Geometry: final body of the model. Coordinates: model frame, mm. A direction names the side the tool comes from. Coordinates: 2 decimals unless noted, no trailing zeros. Order: outer loops, then holes, each group sorted by start corner. A loop starts at its lowest first (then second) coordinate and runs counter-clockwise, first axis right, second up. Notation, with made-up numbers: M 70,-4.5 L 129,-4.5 A14 cw 129,7.5 Z; hole C 34,28.25 d3. An arc over 180 degrees is marked long. Write item = value, one per line.
from build123d import *

# Parameters (mm, degrees)
BOSS_EXTRUDE1_DEPTH = 60
CHAMFER1_SIZE       = 5
SKETCH5_R           = 15
CUT_EXTRUDE1_DEPTH  = 60
CUT_EXTRUDE2_DEPTH  = 60
SKETCH3_R           = 4.5
CUT_EXTRUDE3_DEPTH  = 10


with BuildPart() as part:
    # Sketch1 → Boss-Extrude1 (new body)
    with BuildSketch(Plane.XY):
        with BuildLine():
            Line((0, 0), (0, 174))
            ThreePointArc((0, 174), (2.928932188, 181.071067812), (10, 184))
            Line((10, 184), (60, 184))
            Line((60, 184), (60, 179))
            Line((60, 179), (10, 179))
            ThreePointArc((10, 179), (6.464466094, 177.535533906), (5, 174))
            Line((5, 174), (5, 0))
            Line((5, 0), (0, 0))
        make_face()
    extrude(amount=BOSS_EXTRUDE1_DEPTH)

    # Chamfer1
    chamfer1_edges = [part.edges().sort_by_distance(p)[0] for p in [
        (2.5, 0, 0),
        (2.5, 0, 60),
    ]]
    chamfer(chamfer1_edges, length=CHAMFER1_SIZE)

    # Sketch5 → Cut-Extrude1 (cut)
    with BuildSketch(Plane(origin=(0, 184, 0), x_dir=(1, 0, 0), z_dir=(0, 1, 0))):
        with Locations(Location((40, -30, 0), (0, 0, 270))):
            Circle(SKETCH5_R)
    extrude(amount=-CUT_EXTRUDE1_DEPTH, mode=Mode.SUBTRACT)

    # Sketch6 → Cut-Extrude2 (cut)
    with BuildSketch(Plane(origin=(0, 184, 0), x_dir=(1, 0, 0), z_dir=(0, 1, 0))):
        Polygon((10, 0), (60, -15), (60, 0), align=None)
        Polygon((60, -45), (10, -60), (60, -60), align=None)
    extrude(amount=-CUT_EXTRUDE2_DEPTH, mode=Mode.SUBTRACT)

    # Sketch3 → Cut-Extrude3 (cut)
    with BuildSketch(Plane(origin=(5, 0, 0), x_dir=(0, 0, -1), z_dir=(1, 0, 0))):
        with Locations((-30, 15)):
            Circle(SKETCH3_R)
        with Locations((-30, 75)):
            Circle(SKETCH3_R)
        with Locations((-30, 135)):
            Circle(SKETCH3_R)
    extrude(amount=-CUT_EXTRUDE3_DEPTH, mode=Mode.SUBTRACT)


solid = part.part
1) Line query: L1, parallel to Y at x = 1.35, z = 30; L2, parallel to Y at x = 1.1, z = 30; L3, parallel to X at y = 82.5, z = 57. Output: solid intervals per line, ascending.
Numbers:
L1 = 0 to 10.5, 19.5 to 70.5, 79.5 to 130.5, 139.5 to 179.02
L2 = 0 to 10.5, 19.5 to 70.5, 79.5 to 130.5, 139.5 to 178.56
L3 = 0 to 5
2) Section B-B, the plane z = 42. Return loops of the section in (x, y).
Numbers:
outline = M 0,0 L 5,0 L 5,174 A5 cw 10,179 L 31,179 L 31,184 L 10,184 A10 ccw 0,174 Z; M 49,179 L 60,179 L 60,184 L 49,184 Z
3) Section C-C, the plane x = 52. Return loops of the section in (y, z).
Numbers:
outline = M 179,12.6 L 184,12.6 L 184,21 L 179,21 Z; M 179,39 L 184,39 L 184,47.4 L 179,47.4 Z
4) Set-up query: faces 5 (the face through (60, 182, 30)), 6 (the face through (5, 88, 30)). Return all of +Z, -Z, +X, -X, +Y, -Y with unobstructed straight access to the full face (end or side cutting, diameter ignored); none if empty.
Numbers:
face_5 = +Z, -Z, +X, +Y, -Y
face_6 = +Z, -Z, +X, -Y
5) Mould query, pull axis Y, two halves, no side actions, for faces 1 (the face through (24, 179, 30)), 2 (the face through (2.535, 78.794, 27.581)), 3 (the face through (34.65, 181.535, 7.395)), 4 (the face through (2.54, 130.61, 30.98)). Classes: pulls with the +Y half, pulls with the -Y half, needs draft (parallel to the pull), parting line crosses it, or undercut.
Numbers:
face_1 = pulls with the -Y half
face_2 = undercut
face_3 = needs draft
face_4 = undercut
6) Section D-D, the plane z = 30. Return loops of the section in (x, y).
Numbers:
outline = M 0,0 L 5,0 L 5,10.5 L 0,10.5 Z; M 0,19.5 L 5,19.5 L 5,70.5 L 0,70.5 Z; M 0,79.5 L 5,79.5 L 5,130.5 L 0,130.5 Z; M 0,139.5 L 5,139.5 L 5,174 A5 cw 10,179 L 25,179 L 25,184 L 10,184 A10 ccw 0,174 Z; M 55,179 L 60,179 L 60,184 L 55,184 Z
7) Section A-A, the plane y = 135. Return loops of the section in (x, z), and give its area (3 significant figures).
Numbers:
outline = M 0,0 L 5,0 L 5,25.5 L 0,25.5 Z; M 0,34.5 L 5,34.5 L 5,60 L 0,60 Z
area = 255 mm²
8) Pin query (flat end, axial travel): pin 1 (5 mm diameter, centred on x = 26.5, z = 6.5, fed in from -Y); pin 2 (2 mm diameter, centred on y = 86.5, z = 15.5, fed in from +X). Return the tip coordinate at first contact, or that it passes through.
Numbers:
pin_1 = 179
pin_2 = 5
